from build123d import *

# Parameters (mm, degrees)
SKETCH13_R          = 15
BOSS_EXTRUDE6_DEPTH = 5
BOSS_EXTRUDE7_DEPTH = 50
BOSS_EXTRUDE8_START = 50
SKETCH15_R          = 15
BOSS_EXTRUDE8_DEPTH = 5
CUT_EXTRUDE2_DEPTH  = 41.5
FILLET2_R           = 2


with BuildPart() as part:
    # Sketch13 → Boss-Extrude6 (new body)
    with BuildSketch(Plane.XY):
        with BuildLine():
            Line((2.157181952, 24.906757437), (232, 5))
            Line((232, 5), (232, -5))
            Line((232, -5), (2.157181952, -24.906757437))
            ThreePointArc((2.157181952, -24.906757437), (-25, 0), (2.157181952, 24.906757437))
        make_face()
        Circle(SKETCH13_R, mode=Mode.SUBTRACT)
    extrude(amount=BOSS_EXTRUDE6_DEPTH)

    # Sketch14 → Boss-Extrude7 (add)
    with BuildSketch(Plane.XY.offset(5)):
        Polygon((232, 5), (117.078590976, 14.953378719), (54.588884616, 0), (117.078590976, -14.953378719), (232, -5), align=None)
    extrude(amount=BOSS_EXTRUDE7_DEPTH)

    # Sketch15 → Boss-Extrude8 (add)
    with BuildSketch(Plane.XY.offset(5).offset(BOSS_EXTRUDE8_START)):
        with BuildLine():
            Line((117.078590976, 14.953378719), (2.157181952, 24.906757437))
            ThreePointArc((2.157181952, 24.906757437), (-25, 0), (2.157181952, -24.906757437))
            Line((2.157181952, -24.906757437), (117.078590976, -14.953378719))
            Line((117.078590976, -14.953378719), (232, -5))
            Line((232, -5), (232, 5))
            Line((232, 5), (117.078590976, 14.953378719))
        make_face()
        Circle(SKETCH15_R, mode=Mode.SUBTRACT)
    extrude(amount=BOSS_EXTRUDE8_DEPTH)

    # Sketch16 → Cut-Extrude2 (cut, symmetric)
    with BuildSketch(Plane(origin=(0, 0, 0), x_dir=(1, 0, 0), z_dir=(0, 1, 0))):
        Polygon((232, 0), (133.011770042, 0), (232, -20), align=None)
        Polygon((232, -40), (232, -60), (133.011770042, -60), align=None)
    extrude(amount=CUT_EXTRUDE2_DEPTH, both=True, mode=Mode.SUBTRACT)

    # Sketch20 → Revolve4 (revolve)
    with BuildSketch(Plane(origin=(0, 0, 0), x_dir=(1, 0, 0), z_dir=(0, 1, 0))):
        Polygon((232, -30), (232, -20), (250.852474196, 1.265966163), (250.852474196, -30), align=None)
    revolve(axis=Axis((250.852474196, 0, 30), (-1, 0, 0)))

    # Fillet2
    fillet2_edges = [part.edges().sort_by_distance(p)[0] for p in [
        (250.852474196, 0, 61.265966163),
    ]]
    fillet(fillet2_edges, radius=FILLET2_R)


solid = part.part
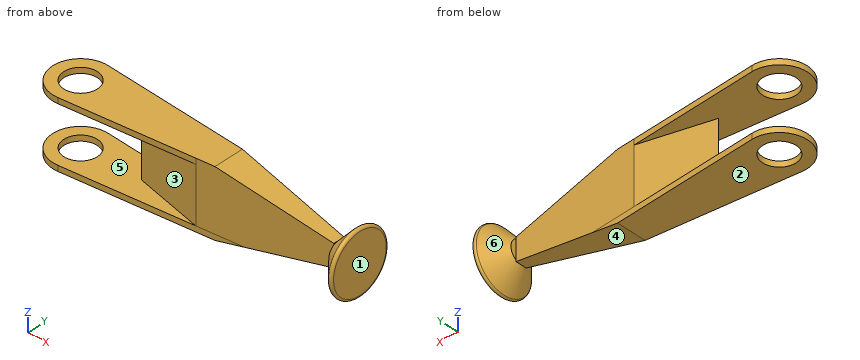
The listing builds one solid part. Answer for the finished solid, in the listing's coordinates (mm). Face numbers are marked on the shaded views. A direction names the side the tool comes from. Give positions to 0.01 mm unless a question says otherwise; leave off trailing zeros. Loops run counter-clockwise (first coordinate to the right, second up) from the corner with the lowest first, then second, coordinate; pieces in that order, holes last.
Item 1: Determine the mould class of the marked faces 1, 2 and 3 for opening direction Z: +Z half, -Z half, draft (parallel to the pull), parting line (faces both ways), or undercut.
Derived:
face 1: draft
face 2: -Z half
face 3: undercut
Item 2: Find the intervals of material crossed by line 1 along Y through (x, z) = (0, 3); line 2 along Z through (x, y) = (-13.5, 14); line 3 along Y through (x, z) = (207, 35), in increasing order.
Derived:
line 1: y = -25 to -15, 15 to 25
line 2: z = 0 to 5, 55 to 60
line 3: y = -7.17 to 7.17
Item 3: A tool of negligible diameter and unlimited length cuts with its end or side. For the marked faces 4, 5 and 6, from which of +Z, -Z, +X, -X, +Y, -Y can it reach the whole face along a straight path? Write none if from no direction.
Derived:
face 4: -Z, +Y, -Y
face 5: -X
face 6: none
Item 4: A cutting plane is placed at C-C (x = 124.5). Give the vertices of the cut face in (y, z), then the cut area to 3 significant figures.
Derived:
outline: (-14.31, 0) - (14.31, 0) - (14.31, 60) - (-14.31, 60) - close
area: 1,720 mm2
Item 5: A cutting plane is placed at B-B (x = 38.5). Give the vertices of the cut face in (y, z).
Derived:
outline: (-21.76, 0) - (21.76, 0) - (21.76, 5) - (-21.76, 5) - close; (-21.76, 55) - (21.76, 55) - (21.76, 60) - (-21.76, 60) - close
Item 6: Each of these flat-tipped pins is pushed along its axis until it touches: pin 1 Ø8 at (x, y) = (190, -1.5) entering from +Z; pin 2 Ø25 at (x, y) = (59.5, 10.5) entering from -Z; pin 3 Ø4 at (x, z) = (119.5, 34) entering from -Y; pin 4 Ø10 at (x, z) = (11, 53.5) entering from +Y. Where does it stop, or does it pass through?
Derived:
pin 1: stops at z = 49.29
pin 2: stops at z = 0
pin 3: stops at y = -14.92
pin 4: stops at y = 24.55
Item 7: A cutting plane is placed at A-A (z = 30). Give the vertices of the cut face in (x, y), then the cut area to 3 significant figures.
Derived:
outline: (54.59, 0) - (117.08, -14.95) - (232, -5) - (232, -10) - (247.36, -27.32) arc R2 ccw to (250.85, -26) - (250.85, 26) arc R2 ccw to (247.36, 27.32) - (232, 10) - (232, 5) - (117.08, 14.95) - close
area: 3,990 mm2
Item 8: A cutting plane is placed at D-D (y = 21.5). Give the number of separate pieces and of enclosed holes in the cut face, then the cut area to 3 significant figures.
Derived:
separate pieces: 3
enclosed holes: 0
area: 777 mm2
